Geometry check sheet. Reference: the model listing, model coordinates, mm. A direction names the side the tool comes from. Give positions to 0.01 mm unless a question says otherwise; leave off trailing zeros. Order: outer loops, then holes, each group sorted by start corner. A loop starts at its lowest first (then second) coordinate and runs counter-clockwise, first axis right, second up. Notation, with made-up numbers: M 80.5,-21 L 117.5,-21 A15 cw 117.5,-12 Z; hole C 72.5,-15 d4. An arc over 180 degrees is marked long. Answer as CSV lines item,"result". Start each with the question number.
Q1. Section check D-D, the plane x = 6.5. Record the boundary of the cut face in (y, z), then the cut area to 3 significant figures.
Q2. Mould release check, pull along Z, two halves, no side actions. Record for faces 4 (the flat face through (12, 2, 1.4)), 5 (the flat face through (2, 2, 0)), 6 (the flat face through (12, 2, -1.4)): +Z half, -Z half, draft (parallel to the pull), parting line (faces both ways), or undercut.
Q3. Thickness scan on line 1 (X direction, y = 2.3, z = 0); line 2 (X direction, y = 1.5, z = -0.3); line 3 (Z direction, x = 16.5, y = 2.1). Record the ranges inside material, lowest first.
Q4. Set-up check for faces 1 (the flat face through (12, 2.5, 0)), 2 (the cylindrical face through (3.24, 2.25, -0.16)), 3 (the flat face through (24.5, 1.3, 0.9)): record each of +Z, -Z, +X, -X, +Y, -Y from which the full face is reachable in a straight line by a thin tool's end or side.
Q5. Section check C-C, the plane y = 0. Record the boundary of the cut face in (x, z), then the cut area to 3 significant figures.
Q6. Section check A-A, the plane x = 2. Record the boundary of the cut face in (y, z), then the cut area to 3 significant figures.
Q7. Section check B-B, the plane z = 0. Record the boundary of the cut face in (x, y).
```python
from build123d import *

# Parameters (mm, degrees)
BOSS_EXTRUDE1_DEPTH = 24.5
SKETCH2_R           = 1.35
BOSS_EXTRUDE2_DEPTH = 10
SKETCH3_R           = 1.25
CUT_EXTRUDE1_DEPTH  = 0.5


with BuildPart() as part:
    # Sketch1 → Boss-Extrude1 (new body)
    with BuildSketch(Plane(origin=(0, 0, 0), x_dir=(0, 0, -1), z_dir=(1, 0, 0))):
        with BuildLine():
            Line((1.4, 1.428285686), (1.4, 2.5))
            Line((1.4, 2.5), (-1.4, 2.5))
            Line((-1.4, 2.5), (-1.4, 1.428285686))
            ThreePointArc((-1.4, 1.428285686), (0, -2), (1.4, 1.428285686))
        make_face()
    extrude(amount=BOSS_EXTRUDE1_DEPTH)

    # Sketch2 → Boss-Extrude2 (add)
    with BuildSketch(Plane(origin=(24.5, 0, 0), x_dir=(0, 0, -1), z_dir=(1, 0, 0))):
        Circle(SKETCH2_R)
    extrude(amount=BOSS_EXTRUDE2_DEPTH)

    # Sketch3 → Cut-Extrude1 (cut)
    with BuildSketch(Plane(origin=(0, 2.5, 0), x_dir=(-1, 0, 0), z_dir=(0, 1, 0))):
        with Locations(Location((-2, 0, 0), (0, 0, 90))):
            Circle(SKETCH3_R)
    extrude(amount=-CUT_EXTRUDE1_DEPTH, mode=Mode.SUBTRACT)


solid = part.part
```
Answer block:
1,outline,"M 1.43,-1.4 L 2.5,-1.4 L 2.5,1.4 L 1.43,1.4 A2 ccw long Z"
1,area,"14.5 mm2"
2,face 4,"+Z half"
2,face 5,"undercut"
2,face 6,"-Z half"
3,line 1,"x = 0 to 0.75, 3.25 to 24.5"
3,line 2,"x = 0 to 24.5"
3,line 3,"z = -1.4 to 1.4"
4,face 1,"+Z, -Z, +X, -X, +Y"
4,face 2,"+Y"
4,face 3,"+X"
5,outline,"M 0,-2 L 24.5,-2 L 24.5,-1.35 L 34.5,-1.35 L 34.5,1.35 L 24.5,1.35 L 24.5,2 L 0,2 Z"
5,area,"125 mm2"
6,outline,"M 1.43,-1.4 L 2.5,-1.4 L 2.5,-1.25 L 2,-1.25 L 2,1.25 L 2.5,1.25 L 2.5,1.4 L 1.43,1.4 A2 ccw long Z"
6,area,"13.2 mm2"
7,outline,"M 0,-2 L 24.5,-2 L 24.5,-1.35 L 34.5,-1.35 L 34.5,1.35 L 24.5,1.35 L 24.5,2.5 L 3.25,2.5 L 3.25,2 L 0.75,2 L 0.75,2.5 L 0,2.5 Z"
